```python
from build123d import *

# Parameters (mm, degrees)
SKETCH2_W               = 150
SKETCH2_H               = 10
CUT_EXTRUDE1_DEPTH      = 10
CUT_EXTRUDE1_DEPTH_BACK = 10
SKETCH5_R               = 4
BOSS_EXTRUDE3_START     = 70
SKETCH7_R               = 10
BOSS_EXTRUDE3_DEPTH     = 70
SKETCH3_R               = 10
BOSS_EXTRUDE4_DEPTH     = 20
SKETCH8_R               = 8
BOSS_EXTRUDE5_DEPTH     = 20
CHAMFER1_SIZE           = 1
CHAMFER2_SIZE           = 1


with BuildPart() as part:
    # Sketch2 → Revolve4 (revolve)
    with BuildSketch(Plane(origin=(0, 0, 0), x_dir=(0, 0, -1), z_dir=(1, 0, 0)), mode=Mode.PRIVATE) as revolve4_sk:
        with Locations((75, 5)):
            Rectangle(SKETCH2_W, SKETCH2_H)
    revolve(revolve4_sk.sketch.rotate(Axis((0, 0, 0), (0, 0, -1)), 90), axis=Axis((0, 0, 0), (0, 0, -1)))

    # Sketch5 → Cut-Extrude1 (cut, two sides: drawn at the far end of the back side and taken through both)
    with BuildSketch(Plane(origin=(0, 0, 0), x_dir=(0, 0, -1), z_dir=(1, 0, 0)).offset(-CUT_EXTRUDE1_DEPTH_BACK)):
        with Locations(Location((135, 0, 0), (0, 0, 180))):
            Circle(SKETCH5_R)
    extrude(amount=CUT_EXTRUDE1_DEPTH + CUT_EXTRUDE1_DEPTH_BACK, mode=Mode.SUBTRACT)

    # Sketch7 → Boss-Extrude3 (add)
    with BuildSketch(Plane.XY.offset(BOSS_EXTRUDE3_START)):
        Circle(SKETCH7_R)
    extrude(amount=-BOSS_EXTRUDE3_DEPTH)

    # Sketch3 → Boss-Extrude4 (add)
    with BuildSketch(Plane(origin=(0, 0, -150), x_dir=(-1, 0, 0), z_dir=(0, 0, -1))):
        with Locations(Location((0, 0, 0), (0, 0, 180))):
            Circle(SKETCH3_R)
    extrude(amount=BOSS_EXTRUDE4_DEPTH)

    # Sketch8 → Boss-Extrude5 (add)
    with BuildSketch(Plane(origin=(0, 0, -170), x_dir=(-1, 0, 0), z_dir=(0, 0, -1))):
        Circle(SKETCH8_R)
    extrude(amount=BOSS_EXTRUDE5_DEPTH)

    # Chamfer1
    chamfer1_edges = [part.edges().sort_by_distance(p)[0] for p in [
        (8, 0, -190),
    ]]
    chamfer(chamfer1_edges, length=CHAMFER1_SIZE)

    # Chamfer2
    chamfer2_edges = [part.edges().sort_by_distance(p)[0] for p in [
        (-10, 0, -170),
    ]]
    chamfer(chamfer2_edges, length=CHAMFER2_SIZE)


solid = part.part
```
Read the model definition and answer for the solid it produces. Units are mm, in the model's axes. Coordinates: 2 decimals unless noted, no trailing zeros. Loops run counter-clockwise (first coordinate to the right, second up) from the corner with the lowest first, then second, coordinate; pieces in that order, holes last.
(1) The part is cut by section C-C (z = 31.5). Determine the outline of the cut face in (x, y), and give its area (3 significant figures).
Solution:
outline: circle Ø20 at (0, 0)
area: 314 mm2
(2) Consider line 1 along Y through (x, z) = (-6, -135); line 2 along Y through (x, z) = (4.5, -135); line 3 along X through (y, z) = (-6, -44). Determine where each line is inside the solid, lowest interval first.
Solution:
line 1: y = -8 to -4, 4 to 8
line 2: y = -8.93 to -4, 4 to 8.93
line 3: x = -8 to 8
(3) The part is cut by section D-D (z = -135). Determine the outline of the cut face in (x, y), and give its area (3 significant figures).
Solution:
outline: (-9.17, -4) arc R10 ccw to (9.17, -4) - close; (-9.17, 4) - (9.17, 4) arc R10 ccw to start
area: 159 mm2
(4) Flat-ended cylindrical pins translate along their axes: pin 1 Ø5 at (y, z) = (0, -135) entering from +X; pin 2 Ø1.5 at (y, z) = (4, -10) entering from +X; pin 3 Ø1 at (x, y) = (-8, -6.5) entering from -Z. Find the tip coordinate at first contact, or state that the pin passes through.
Solution:
pin 1: passes through
pin 2: stops at x = 9.46
pin 3: stops at z = -169.19
(5) The part is cut by section A-A (y = 0). Determine the outline of the cut face in (x, z), and give its area (3 significant figures).
Solution:
outline: (-10, -169) - (-9, -170) - (-8, -170) - (-8, -189) - (-7, -190) - (7, -190) - (8, -189) - (8, -170) - (9, -170) - (10, -169) - (10, -139) - (-10, -139) - close; (-10, -131) - (10, -131) - (10, 70) - (-10, 70) - close
area: 4,960 mm2
(6) The part is cut by section B-B (x = 0). Determine the outline of the cut face in (y, z), and give its area (3 significant figures).
Solution:
outline: (-10, -169) - (-9, -170) - (-8, -170) - (-8, -189) - (-7, -190) - (7, -190) - (8, -189) - (8, -170) - (9, -170) - (10, -169) - (10, 70) - (-10, 70) - close; hole circle Ø8 at (0, -135)
area: 5,070 mm2
(7) The mould has two halves that part along Y. Classify faces 1 (the face through (1.73, -7.81, -179.37)), 2 (the face through (0, 0, -190)), 3 (the face through (-0.14, -1.201, -131.185)): released by +Y, released by -Y, zero draft, split by the parting line, or undercut.
Solution:
face 1: split by the parting line
face 2: zero draft
face 3: undercut
